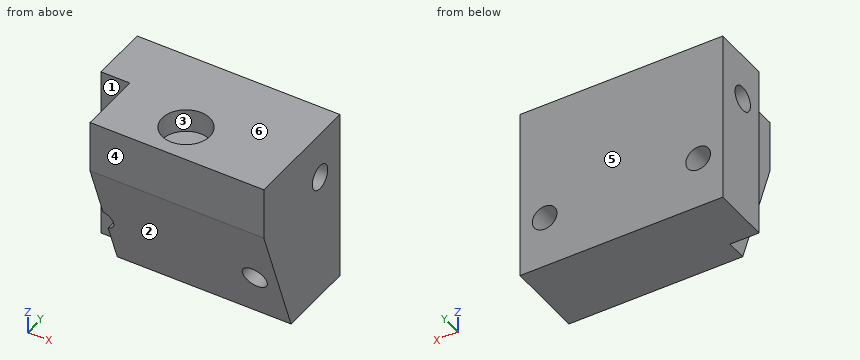
```python
from build123d import *

# Parameters (mm, degrees)
SKETCH1_W           = 70
SKETCH1_H           = 60
BOSS_EXTRUDE1_DEPTH = 20
BOSS_EXTRUDE2_DEPTH = 60
SKETCH5_R           = 4.25
CUT_EXTRUDE3_DEPTH  = 131
SKETCH7_R           = 4.25
CUT_EXTRUDE4_DEPTH  = 91
SKETCH8_R           = 8.25
CUT_EXTRUDE5_DEPTH  = 8


with BuildPart() as part:
    # Sketch1 → Boss-Extrude1 (new body)
    with BuildSketch(Plane(origin=(0, 0, 0), x_dir=(1, 0, 0), z_dir=(0, 1, 0))):
        Rectangle(SKETCH1_W, SKETCH1_H)
    extrude(amount=BOSS_EXTRUDE1_DEPTH)

    # Sketch2 → Boss-Extrude2 (add)
    with BuildSketch(Plane(origin=(35, 0, 0), x_dir=(0, 0, -1), z_dir=(1, 0, 0))):
        Polygon((30, 20), (30, 0), (30, -7), (-12, -22), (-30, -22), (-30, 20), align=None)
    extrude(amount=-BOSS_EXTRUDE2_DEPTH)

    # Sketch5 → Cut-Extrude3 (cut)
    with BuildSketch(Plane.ZY.offset(35)):
        with Locations((14, 9)):
            Circle(SKETCH5_R)
    extrude(amount=-CUT_EXTRUDE3_DEPTH, mode=Mode.SUBTRACT)

    # Sketch7 → Cut-Extrude4 (cut)
    with BuildSketch(Plane(origin=(0, 20, 0), x_dir=(1, 0, 0), z_dir=(0, 1, 0))):
        with Locations(Location((26.5, 12, 0), (0, 0, 270))):
            Circle(SKETCH7_R)
        with Locations(Location((-26.5, 12, 0), (0, 0, 290.667316494))):
            Circle(SKETCH7_R)
    extrude(amount=-CUT_EXTRUDE4_DEPTH, mode=Mode.SUBTRACT)

    # Sketch8 → Cut-Extrude5 (cut)
    with BuildSketch(Plane.XY.offset(30)):
        with Locations((0, -9)):
            Circle(SKETCH8_R)
    extrude(amount=-CUT_EXTRUDE5_DEPTH, mode=Mode.SUBTRACT)


solid = part.part
```
Could you check a few things on this model? Use its own coordinates, in mm. Face numbers are marked on the shaded views. A direction names the side the tool comes from. Give positions to 0.01 mm unless a question says otherwise; leave off trailing zeros. Write each loop counter-clockwise with the first axis right and the second up, starting at its lowest first coordinate (ties: lowest second). Pieces come first, ordered by that corner, then holes. Notation, with made-up numbers: (-25, 81.25) - (21, 81.25) arc R17 ccw to (21, 106.25) - close; hole circle Ø6 at (50, -24.75). An arc over 180 degrees is marked (long way). One line per item, written item: value. Start each with the question number.
Item 1: Please list where these lines run through material, in increasing order: line 1 (X direction, y = 3, z = -12); line 2 (X direction, y = -3, z = -12); line 3 (Z direction, x = 26.5, y = 12.5). Write a range as from..to.
Item 2: Which directions (+Z, -Z, +X, -X, +Y, -Y) give clear straight access to the entire face, cutting with the end or side of a thin tool? Please do the marked faces 1 and 2.
Item 3: Imagine slicing it at C-C, the plane y = -9. List the corners of the cut face in (x, z) for me.
Item 4: I'm going to push flat-ended pins straight in: pin 1 (6 mm diameter, centred on y = -3.5, z = -24, fed in from -X); pin 2 (6 mm diameter, centred on x = -7.5, z = -23.5, fed in from -Y). Where does each tip first touch, or does it pass through?
Item 5: If we mould it in two halves opening along Y, with no side actions, what happens to the marked faces 3, 4, 5 and 6? For each: +Y half, -Y half, draft (parallel to the pull), parting line (faces both ways), or undercut.
Item 6: Imagine slicing it at A-A, the plane x = -26.5. List the corners of the cut face in (y, z) for me.
Item 7: Imagine slicing it at D-D, the plane x = 0. List the corners of the cut face in (y, z) for me, and give its area (3 significant figures).
Item 8: Imagine slicing it at B-B, the plane z = 14. List the corners of the cut face in (x, y) for me.
Geometry says:
1. line 1: -35..-30.75, -22.25..22.25, 30.75..35
1. line 2: -22.25..22.25, 30.75..35
1. line 3: -30..-16.25, -7.75..11.59, 16.41..30
2. face 1: +Z, -Z, -X, -Y
2. face 2: -Z, +X, -X, -Y
3. outline: (-25, -24.4) - (35, -24.4) - (35, 30) - (8.25, 30) - (8.25, 22) - (-8.25, 22) - (-8.25, 30) - (-25, 30) - (-25, -8.02) arc R4.25 cw to (-25, -15.98) - close; hole circle Ø8.5 at (26.5, -12)
4. pin 1: x = -25
4. pin 2: y = -10.39
5. face 3: undercut
5. face 4: -Y half
5. face 5: +Y half
5. face 6: draft
6. outline: (0, -30) - (20, -30) - (20, -16.25) - (0, -16.25) - close; (0, -7.75) - (20, -7.75) - (20, 30) - (0, 30) - close; hole circle Ø8.5 at (9, 14)
7. outline: (-22, 12) - (-7, -30) - (20, -30) - (20, 30) - (-0.75, 30) - (-0.75, 22) - (-17.25, 22) - (-17.25, 30) - (-22, 30) - close; hole circle Ø8.5 at (9, 14)
7. area: 2,020 mm^2
8. outline: (-35, 0) - (-25, 0) - (-25, -22) - (35, -22) - (35, 4.75) - (-35, 4.75) - close; (-35, 13.25) - (35, 13.25) - (35, 20) - (-35, 20) - close
